from build123d import *

# Parameters (mm, degrees)
SKETCH_1_W          = 530
SKETCH_1_H          = 280
EXTRUDE_1_DEPTH     = 2
SKETCH_2_R          = 10
CUT_EXTRUDE_1_DEPTH = 2
SKETCH_3_W          = 96.084131949
SKETCH_3_H          = 15
SKETCH_3_W_2        = 93.312729878
CUT_EXTRUDE_2_DEPTH = 10


with BuildPart() as part:
    # 草图1 → 凸台-拉伸1 (new body)
    with BuildSketch(Plane(origin=(0, 0, 0), x_dir=(1, 0, 0), z_dir=(0, 1, 0))):
        Rectangle(SKETCH_1_W, SKETCH_1_H)
    extrude(amount=EXTRUDE_1_DEPTH)

    # 草图2 → 切除-拉伸1 (cut)
    with BuildSketch(Plane(origin=(0, 2, 0), x_dir=(1, 0, 0), z_dir=(0, 1, 0))):
        with Locations(Location((-240, 115, 0), (0, 0, 270))):
            Circle(SKETCH_2_R)
        with Locations(Location((-240, -115, 0), (0, 0, 90))):
            Circle(SKETCH_2_R)
        with Locations(Location((240, -115, 0), (0, 0, 270))):
            Circle(SKETCH_2_R)
        with Locations(Location((240, 115, 0), (0, 0, 90))):
            Circle(SKETCH_2_R)
    extrude(amount=-CUT_EXTRUDE_1_DEPTH, mode=Mode.SUBTRACT)

    # 草图3 → 切除-拉伸2 (cut)
    with BuildSketch(Plane(origin=(0, 2, 0), x_dir=(1, 0, 0), z_dir=(0, 1, 0))):
        with Locations((-251.042065975, -28.5)):
            Rectangle(SKETCH_3_W, SKETCH_3_H)
        with Locations((-249.656364939, 48.5)):
            Rectangle(SKETCH_3_W_2, SKETCH_3_H)
    extrude(amount=-CUT_EXTRUDE_2_DEPTH, mode=Mode.SUBTRACT)


solid = part.part
Check sheet for the modelled part. Datum: model origin and axes. Units: mm. Round coordinates to 2 decimals unless told otherwise and drop trailing zeros. Order: outer loops, then holes, each group sorted by start corner. A loop starts at its lowest first (then second) coordinate and runs counter-clockwise, first axis right, second up.
Q1. Depth check by flat-ended pin: P1, Ø1, axis at y = 1, z = -51, coming from the -X side. Enter the tip coordinate at first touch or a pass-through.
Filled sheet:
P1: stops at x = -203
Q2. Scan lines: L1, parallel to Z at x = -204, y = 1.15; L2, parallel to X at y = 0.7, z = -115; L3, parallel to X at y = 0.3, z = 112. Record each from-to range of solid material in increasing order.
Filled sheet:
L1: z = -140 to -56, -41 to 21, 36 to 140
L2: x = -265 to -250, -230 to 230, 250 to 265
L3: x = -265 to -249.54, -230.46 to 230.46, 249.54 to 265
Q3. Cross-section at B-B, the plane z = 115. Enter the section's corners in (x, y).
Filled sheet:
outline: (-265, 0) - (-250, 0) - (-250, 2) - (-265, 2) - close; (-230, 0) - (230, 0) - (230, 2) - (-230, 2) - close; (250, 0) - (265, 0) - (265, 2) - (250, 2) - close
Q4. Cross-section at A-A, the plane x = 240. Enter the section's corners in (y, z), plus the area to 3 significant figures.
Filled sheet:
outline: (0, -140) - (2, -140) - (2, -125) - (0, -125) - close; (0, -105) - (2, -105) - (2, 105) - (0, 105) - close; (0, 125) - (2, 125) - (2, 140) - (0, 140) - close
area: 480 mm2
Q5. Cross-section at C-C, the plane x = -240. Enter the section's corners in (y, z), plus the area to 3 significant figures.
Filled sheet:
outline: (0, -140) - (2, -140) - (2, -125) - (0, -125) - close; (0, -105) - (2, -105) - (2, -56) - (0, -56) - close; (0, -41) - (2, -41) - (2, 21) - (0, 21) - close; (0, 36) - (2, 36) - (2, 105) - (0, 105) - close; (0, 125) - (2, 125) - (2, 140) - (0, 140) - close
area: 420 mm2
Q6. Draft check along X on faces 1 (the face through (246.76, 1.01, 107.63)), 2 (the face through (233.24, 1.01, -107.63)), 3 (the face through (-4, 2, -2)). Enter one of: pulls with the +X half, pulls with the -X half, needs draft (parallel to the pull), parting line crosses it, or undercut.
Filled sheet:
face 1: undercut
face 2: undercut
face 3: needs draft
Q7. Cross-section at D-D, the plane y = 0.45. Enter the section's corners in (x, z).
Filled sheet:
outline: (-265, -140) - (265, -140) - (265, 140) - (-265, 140) - (-265, 36) - (-203, 36) - (-203, 21) - (-265, 21) - (-265, -41) - (-203, -41) - (-203, -56) - (-265, -56) - close; hole circle Ø20 at (-240, -115); hole circle Ø20 at (-240, 115); hole circle Ø20 at (240, -115); hole circle Ø20 at (240, 115)
